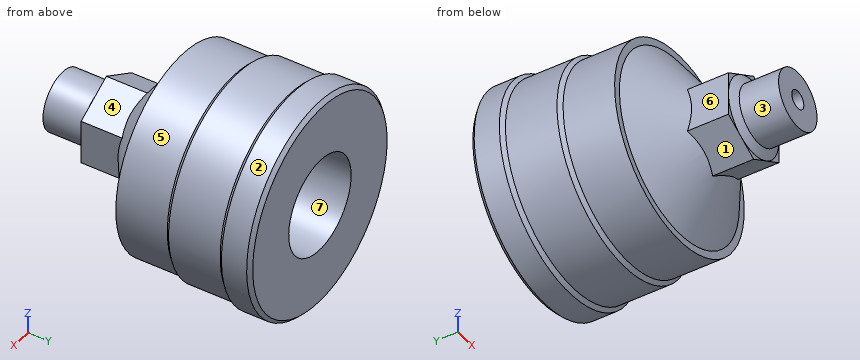
from build123d import *

# Parameters (mm, degrees)
EXTRUDE1_DEPTH = 20.153009


with BuildPart() as part:
    # Sketch1 → Revolve1 (revolve)
    with BuildSketch(Plane.XY, mode=Mode.PRIVATE) as revolve1_sk:
        Polygon((-28, 70), (-29, 69), (-29, 62.153009304), (-28, 61.153009304), (-28, 47.153009304), (-27, 46.153009304), (-27, 32.153009304), (-25, 32.153009304), (-10.5, 22), (-10.5, 12), (-8, 10.698582374), (-8, 0), (-2.5, 0), (-2.5, 32.153009304), (-13.003113073, 47.153009304), (-13.003113073, 70), align=None)
    revolve(revolve1_sk.sketch.rotate(Axis((0, 0, 0), (0, -1, 0)), 270), axis=Axis((0, 0, 0), (0, -1, 0)))

    # Sketch2 → Extrude1 (add)
    with BuildSketch(Plane(origin=(0, 12, 0), x_dir=(-1, 0, 0), z_dir=(0, 1, 0))):
        Polygon((-10.5, 6.062177826), (-10.5, -6.062177826), (0, -12.124355653), (10.5, -6.062177826), (10.5, 6.062177826), (0, 12.124355653), align=None)
    extrude(amount=EXTRUDE1_DEPTH)


solid = part.part
The model under review builds one solid part; all positions refer to its coordinate system, in mm. Face numbers are marked on the shaded views. A direction names the side the tool comes from. Round coordinates to 2 decimals unless told otherwise and drop trailing zeros. Loops run counter-clockwise (first coordinate to the right, second up) from the corner with the lowest first, then second, coordinate; pieces in that order, holes last. Notation, with made-up numbers: (-11, -32.5) -> (39, -32.5) arc R16 cw to (39, -21.5) -> close; hole circle Ø9 at (-7.5, 31.25). An arc over 180 degrees is marked (long way). Answer as CSV lines item,"result".
1) Draft analysis for pull direction Z (two halves, no side actions). For the marked faces 5, 6 and 7, state which applies: pulls with the +Z half, pulls with the -Z half, needs draft (parallel to the pull), parting line crosses it, or undercut.
Geometry results:
face 5,"parting line crosses it"
face 6,"needs draft"
face 7,"undercut"
2) Add section A-A on y = 54.5. Write out the cut boundary in (x, z).
Geometry results:
outline,"circle Ø56 at (0, 0); hole circle Ø26.01 at (0, 0)"
3) Add section B-B on y = 16. Write out the cut boundary in (x, z).
Geometry results:
outline,"(-10.5, -6.06) -> (0, -12.12) -> (10.5, -6.06) -> (10.5, 6.06) -> (0, 12.12) -> (-10.5, 6.06) -> close"
4) For P1, Ø4, axis at x = 0, z = 0, coming from the +Y side; P2, Ø12, axis at x = -18.5, y = 37, coming from the +Z side; P3, Ø9, axis at y = 15, z = 2.5, coming from the +X side, all flat-tipped, find the tip position at first contact; note any pin that passes through.
Geometry results:
P1,"stops at y = 32.15"
P2,"stops at z = 23.93"
P3,"stops at x = 10.5"
5) Tool access review of the marked faces 1, 2, 3 and 4: name each direction out of +Z, -Z, +X, -X, +Y, -Y from which nothing blocks a thin tool from reaching the whole face with its end or side.
Geometry results:
face 1,"-Z, -X, -Y"
face 2,"+Y, -Y"
face 3,"-Y"
face 4,"+Z, +X, -Y"
6) To check wall thickness, follow line 1 along X through (y, z) = (5, 0); line 2 along X through (y, z) = (51.5, -7); line 3 along Z through (x, y) = (-3, 55). State the ranges of each line that lie inside material, in increasing order. Write a range as from..to.
Geometry results:
line 1,"x = -8..-2.5, 2.5..8"
line 2,"x = -27.11..-10.96, 10.96..27.11"
line 3,"z = -27.84..-12.65, 12.65..27.84"
7) Add section C-C on y = 4. Write out the cut boundary in (x, z), plus the area to 3 significant figures.
Geometry results:
outline,"circle Ø16 at (0, 0); hole circle Ø5 at (0, 0)"
area,"181 mm²"
